Verification items for the finished model (mm, model axes). Coordinates: 2 decimals unless noted, no trailing zeros. Order: outer loops, then holes, each group sorted by start corner. A loop starts at its lowest first (then second) coordinate and runs counter-clockwise, first axis right, second up. Notation, with made-up numbers: M 19,41 L 77,41 A37 cw 77,77 Z; hole C -7.75,84 d5. An arc over 180 degrees is marked long. Answer as a JSON object with one key per item and string values. Group by question number.
(1) Cross-section at A-A (z = 4.75). Enter the section's corners in (x, y), plus the area to 3 significant figures.
(2) Material ranges on line 1 (Y direction, x = 1520, z = 12.5); line 2 (X direction, y = 168, z = 15); line 3 (Y direction, x = 1520, z = 9.5), recorded low to high.
(3) Mould release check, pull along Y, two halves, no side actions. Record for faces 1 (the face through (1072, 700, 25)), 2 (the face through (759.1, 104.2, 9.4)): released by +Y, released by -Y, zero draft, split by the parting line, or undercut.
(4) Cross-section at B-B (x = 1377.5). Enter the section's corners in (y, z).
(5) Cross-section at C-C (y = 1275.5). Enter the section's corners in (x, z).
(6) Gauge pin test, flat ends, axial feed: pin 1 Ø7.5 at (y, z) = (1261.5, 18) entering from +X; pin 2 Ø8 at (x, z) = (1036, 12.5) entering from +Y; pin 3 Ø12 at (x, z) = (1101, 3) entering from -Y. Record the tip position at first contact, or that the pin passes through.
from build123d import *

# Parameters (mm, degrees)
SKETCH1_R            = 485
BOSS_EXTRUDE1_DEPTH  = 25
CHAMFER1_SIZE        = 10
M20_THREADED_HOLE1_D = 17.5


with BuildPart() as part:
    # Sketch1 → Boss-Extrude1 (new body)
    with BuildSketch(Plane.XY):
        Polygon((0, 0), (1775, 0), (1775, 1110), (605, 1110), (605, 1380), (0, 1380), align=None)
        with Locations((535, 535)):
            Circle(SKETCH1_R, mode=Mode.SUBTRACT)
    extrude(amount=BOSS_EXTRUDE1_DEPTH)

    # Chamfer1
    chamfer1_edges = [part.edges().sort_by_distance(p)[0] for p in [
        (50, 535, 0),
        (1775, 555, 0),
        (887.5, 0, 0),
        (0, 690, 0),
    ]]
    chamfer(chamfer1_edges, length=CHAMFER1_SIZE)

    # M20 Threaded hole1 (through all)
    with Locations(Plane(origin=(1520, 215, 0), x_dir=(-1, 0, 0), z_dir=(0, 0, -1))):
        with Locations((0, 0), (0, -50)):
            Hole(M20_THREADED_HOLE1_D / 2)


solid = part.part
Taken from the geometry:
{
 "1": {"outline": "M 5.25,5.25 L 1769.75,5.25 L 1769.75,1110 L 605,1110 L 605,1380 L 5.25,1380 Z; hole C 535,535 d980.5; hole C 1520,165 d17.5; hole C 1520,215 d17.5", "area": "1,360,000 mm²"},
 "2": {"line 1": "y = 0 to 156.25, 173.75 to 206.25, 223.75 to 1110", "line 2": "x = 0 to 217.93, 852.07 to 1511.78, 1528.22 to 1775", "line 3": "y = 0.5 to 156.25, 173.75 to 206.25, 223.75 to 1110"},
 "3": {"face 1": "zero draft", "face 2": "undercut"},
 "4": {"outline": "M 0,10 L 10,0 L 1110,0 L 1110,25 L 0,25 Z"},
 "5": {"outline": "M 0,10 L 10,0 L 605,0 L 605,25 L 0,25 Z"},
 "6": {"pin 1": "stops at x = 605", "pin 2": "stops at y = 1110", "pin 3": "stops at y = 1"}
}
